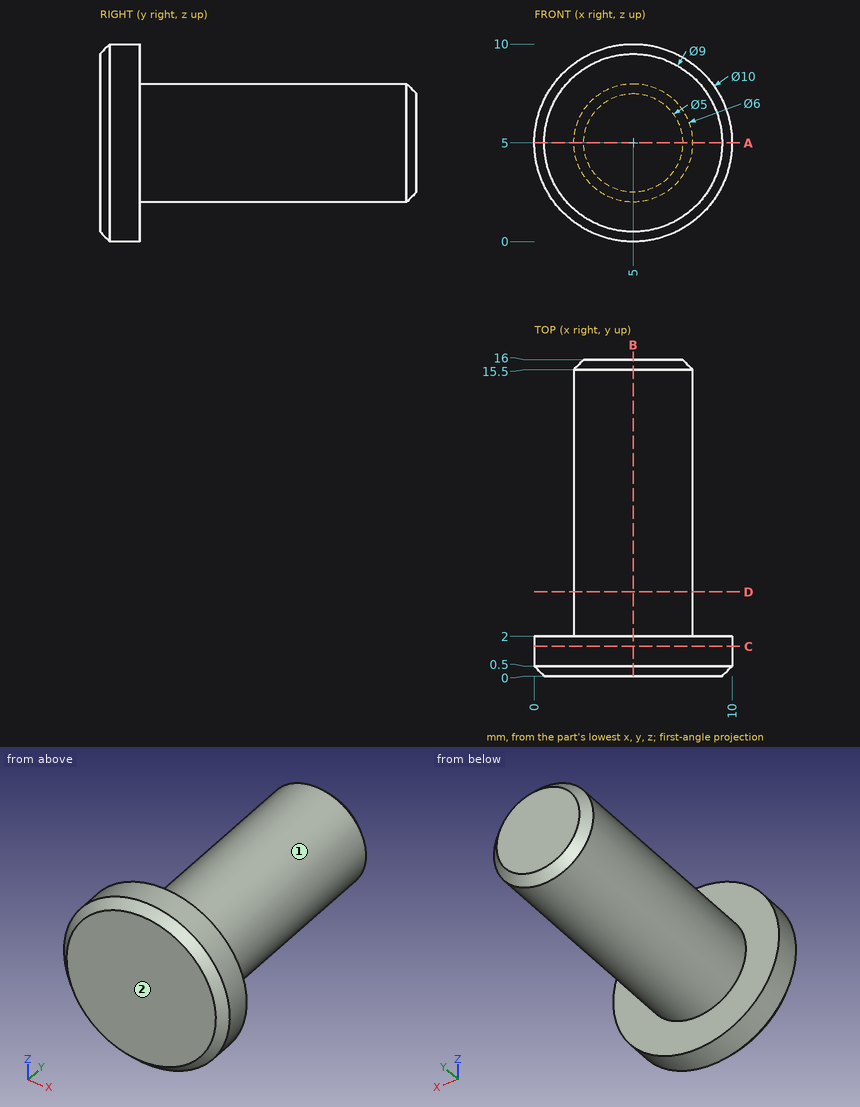
Study the drawing (mm; zero at the part's minimum x, y, z) and answer. A direction names the side the tool comes from. Give positions to 0.01 mm unless a question says otherwise; leave off trailing zeros. Order: outer loops, then holes, each group sorted by start corner. A loop starts at its lowest first (then second) coordinate and runs counter-clockwise, first axis right, second up. Notation, with made-up numbers: (-38.5, 87) - (14.5, 87) arc R14 cw to (14.5, 109) - close; hole circle Ø4 at (35.25, -4). An arc over 180 degrees is marked (long way). Answer in a Markdown table with one row per item. Add a question column.
Q1. Find the intervals of material crossed by line 1 along Y through (x, z) = (2.5, 7); line 2 along Y through (x, z) = (3, 0.5); line 3 along X through (y, z) = (8.5, 5), in increasing order. Write a range as [from, to].
Q2. The part is cut by section D-D (y = 4.25). Determine the outline of the cut face in (x, z), then the cut area to 3 significant figures.
Q3. Which of the six approach directions +Z, -Z, +X, -X, +Y, -Y give full straight-line access (tool end or side, diameter ignored) to the marked faces 1 and 2?
Q4. The part is cut by section A-A (z = 5). Determine the outline of the cut face in (x, y), then the cut area to 4 significant figures.
Q5. The part is cut by section C-C (y = 1.5). Determine the outline of the cut face in (x, z), then the cut area to 3 significant figures.
Q6. The part is cut by section B-B (x = 5). Determine the outline of the cut face in (y, z), then the cut area to 4 significant figures.
Q7. Given P1, Ø2, axis at y = 13, z = 7.5, coming from the -X side; P2, Ø3, axis at x = 4.5, y = 14.5, coming from the +Z side; P3, Ø1, axis at x = 5.5, z = 2, coming from the +Y side, each flat-ended and moving along its own axis, determine where each tip first touches the part or whether it passes through.
Determined:
| question | item | result |
|---|---|---|
| 1 | line 1 | y = [0, 2] |
| 1 | line 2 | y = [0.42, 2] |
| 1 | line 3 | x = [2, 8] |
| 2 | outline | circle Ø6 at (5, 5) |
| 2 | area | 28.3 mm² |
| 3 | face 1 | +Y |
| 3 | face 2 | +Z, -Z, +X, -X, -Y |
| 4 | outline | (0, 0.5) - (0.5, 0) - (9.5, 0) - (10, 0.5) - (10, 2) - (8, 2) - (8, 15.5) - (7.5, 16) - (2.5, 16) - (2, 15.5) - (2, 2) - (0, 2) - close |
| 4 | area | 103.5 mm² |
| 5 | outline | circle Ø10 at (5, 5) |
| 5 | area | 78.5 mm² |
| 6 | outline | (0, 0.5) - (0.5, 0) - (2, 0) - (2, 2) - (15.5, 2) - (16, 2.5) - (16, 7.5) - (15.5, 8) - (2, 8) - (2, 10) - (0.5, 10) - (0, 9.5) - close |
| 6 | area | 103.5 mm² |
| 7 | P1 | stops at x = 2.4 |
| 7 | P2 | stops at z = 8 |
| 7 | P3 | stops at y = 15.96 |
